```python
from build123d import *

# Parameters (mm, degrees)
SKETCH1_R                                            = 25
BOSS_EXTRUDE1_DEPTH                                  = 6
HOLE_SIZE_BASED_ON_SOCKET_HEAD_CAP_SCREW_D           = 4.5
HOLE_SIZE_BASED_ON_SOCKET_HEAD_CAP_SCREW_DEPTH       = 10.1
HOLE_SIZE_BASED_ON_SOCKET_HEAD_CAP_SCREW_CBORE_D     = 8
HOLE_SIZE_BASED_ON_SOCKET_HEAD_CAP_SCREW_CBORE_DEPTH = 4.6
HOLE_SIZE_BASED_ON_SOCKET_HEAD_CAP_SCREW_TIP         = 1.351936393


with BuildPart() as part:
    # Sketch1 → Boss-Extrude1 (new body)
    with BuildSketch(Plane(origin=(0, 0, 0), x_dir=(1, 0, 0), z_dir=(0, 1, 0))):
        with Locations(Location((0, 0, 0), (0, 0, 270))):
            Circle(SKETCH1_R)
    extrude(amount=BOSS_EXTRUDE1_DEPTH)

    # Hole size based on socket head cap screw type 1
    with Locations(Plane(origin=(16.864722122, 6, -0.289543132), x_dir=(0, 0, 1), z_dir=(0, 1, 0))):
        with Locations((0, 0), (0.961754182, -34.5679876)):
            CounterBoreHole(HOLE_SIZE_BASED_ON_SOCKET_HEAD_CAP_SCREW_D / 2, HOLE_SIZE_BASED_ON_SOCKET_HEAD_CAP_SCREW_CBORE_D / 2, HOLE_SIZE_BASED_ON_SOCKET_HEAD_CAP_SCREW_CBORE_DEPTH, depth=HOLE_SIZE_BASED_ON_SOCKET_HEAD_CAP_SCREW_DEPTH)
            with Locations((0, 0, -(HOLE_SIZE_BASED_ON_SOCKET_HEAD_CAP_SCREW_DEPTH + HOLE_SIZE_BASED_ON_SOCKET_HEAD_CAP_SCREW_TIP / 2))):  # 118° drill point
                Cone(0, HOLE_SIZE_BASED_ON_SOCKET_HEAD_CAP_SCREW_D / 2, HOLE_SIZE_BASED_ON_SOCKET_HEAD_CAP_SCREW_TIP, mode=Mode.SUBTRACT)


solid = part.part
```
Part model, mm, in its own coordinate system. A direction names the side the tool comes from. Round coordinates to 2 decimals unless told otherwise and drop trailing zeros. Write each loop counter-clockwise with the first axis right and the second up, starting at its lowest first coordinate (ties: lowest second). Pieces come first, ordered by that corner, then holes. Notation, with made-up numbers: M 87.25,85.5 L 91.25,85.5 A26 ccw 91.25,121.5 Z; hole C 1.5,4.5 d2. An arc over 180 degrees is marked long. Answer as CSV lines item,"result". Start each with the question number.
1) Which spindle directions (+Z, -Z, +X, -X, +Y, -Y) get a long thin tool onto all of the face, cutting with end or side? Do faces 4 (the face through (-21.25, 3.73, 2.52)), 5 (the face through (0, 6, 0)). Say none if no direction does.
2) Band-saw the part on D-D (x = -12). List the corners of the cut face in (y, z), then the cut area to 3 significant figures.
3) Band-saw the part on A-A (z = -1). List the corners of the cut face in (x, y).
4) Drill centre lines: L1, parallel to X at y = 5, z = 1; L2, parallel to Z at x = 20, y = 5.7; L3, parallel to Z at x = -20, y = 1.45. Where is each one in solid material? Low to high.
5) Band-saw the part on B-B (x = 20). List the corners of the cut face in (y, z), then the cut area to 3 significant figures.
6) Band-saw the part on C-C (y = 3.15). List the corners of the cut face in (x, z).
7) Mould opens along Z. For faces 1 (the face through (7.509, 2.958, 23.846)), 2 (the face through (-15.472, 0.69, 0.965)), 3 (the face through (0, 0, 0)) say: +Z half, -Z half, draft (parallel to the pull), parting line (faces both ways), or undercut.
8) Drop flat-ended pins along their axis: pin 1 (2 mm diameter, centred on x = 15.5, y = 3, fed in from +Z); pin 2 (2.5 mm diameter, centred on x = 18, z = 0, fed in from +Y). Give the stop position or say it passes through.
Worked out:
1,face 4,"+Y"
1,face 5,"+Z, -Z, +X, -X, +Y"
2,outline,"M 0,-21.93 L 6,-21.93 L 6,21.93 L 0,21.93 Z"
2,area,"263 mm²"
3,outline,"M -24.98,0 L -19.21,0 L -19.21,1.4 L -21.34,1.4 L -21.34,6 L -24.98,6 Z; M -16.2,0 L 14.73,0 L 14.73,1.4 L 12.93,1.4 L 12.93,6 L -14.07,6 L -14.07,1.4 L -16.2,1.4 Z; M 19,0 L 24.98,0 L 24.98,6 L 20.8,6 L 20.8,1.4 L 19,1.4 Z"
4,L1,"-24.98 to -21.69, -13.72 to 13.08, 20.65 to 24.98"
4,L2,"-15 to -2.77, 2.19 to 15"
4,L3,"-15 to -2.6, 3.95 to 15"
5,outline,"M 0,-15 L 6,-15 L 6,-2.77 L 1.4,-2.77 L 1.4,2.19 L 6,2.19 L 6,15 L 0,15 Z"
5,area,"157 mm²"
6,outline,"C 0,0 d50; hole C -17.7,0.67 d8; hole C 16.86,-0.29 d8"
7,face 1,"parting line"
7,face 2,"undercut"
7,face 3,"draft"
8,pin 1,"z = 20.37"
8,pin 2,"y = 1.4"
